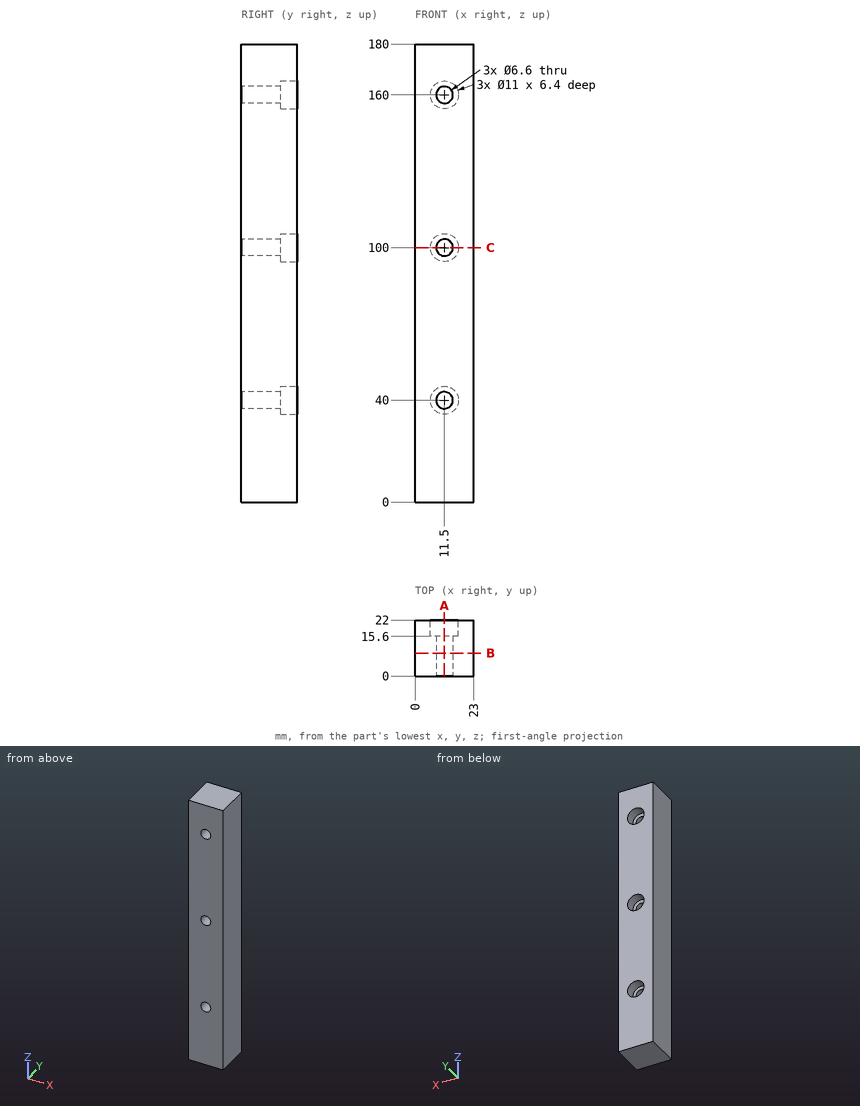
Design review of the part shown in the three views and the two pictorial views. Dimensions are in mm from the part's minimum x, y and z. Give positions to 0.01 mm unless a question says otherwise; leave off trailing zeros. Write each loop counter-clockwise with the first axis right and the second up, starting at its lowest first coordinate (ties: lowest second). Pieces come first, ordered by that corner, then holes. Notation, with made-up numbers: (70.5, 35.5) - (125.5, 35.5) arc R29 ccw to (125.5, 55.5) - close; hole circle Ø6 at (55.25, 61). An arc over 180 degrees is marked (long way). Return JSON: item names as keys, results as strings. Group by question number.
(1) We need section A-A, the plane x = 11.5. Give the boundary of the cut face in (y, z), then the cut area to 3 significant figures.
(2) Insertion check: pin 1 (10 mm diameter, centred on y = 14, z = 109, fed in from -X); pin 2 (5.5 mm diameter, centred on x = 11.5, z = 40, fed in from -Y); pin 3 (10.5 mm diameter, centred on x = 11.5, z = 160, fed in from +Y). Each pin has a flat end and moves straight along its axis. Give the tip position at first contact, or say it passes through.
(3) To check wall thickness, follow probe 1 along Z at (x, y) = (11.5, 12); probe 2 along Z at (x, y) = (11.5, 20); probe 3 along X at (y, z) = (19.75, 100). State the ranges of each line that lie inside material, in increasing order.
(4) We need section C-C, the plane z = 100. Give the boundary of the cut face in (x, y), then the cut area to 3 significant figures.
(5) We need section B-B, the plane y = 9. Give the boundary of the cut face in (x, z), then the cut area to 3 significant figures.
Reported:
{
 "1": {"outline": "(0, 0) - (22, 0) - (22, 34.5) - (15.6, 34.5) - (15.6, 36.7) - (0, 36.7) - close; (0, 43.3) - (15.6, 43.3) - (15.6, 45.5) - (22, 45.5) - (22, 94.5) - (15.6, 94.5) - (15.6, 96.7) - (0, 96.7) - close; (0, 103.3) - (15.6, 103.3) - (15.6, 105.5) - (22, 105.5) - (22, 154.5) - (15.6, 154.5) - (15.6, 156.7) - (0, 156.7) - close; (0, 163.3) - (15.6, 163.3) - (15.6, 165.5) - (22, 165.5) - (22, 180) - (0, 180) - close", "area": "3,440 mm2"},
 "2": {"pin 1": "stops at x = 0", "pin 2": "passes through", "pin 3": "stops at y = 15.6"},
 "3": {"probe 1": "z = 0 to 36.7, 43.3 to 96.7, 103.3 to 156.7, 163.3 to 180", "probe 2": "z = 0 to 34.5, 45.5 to 94.5, 105.5 to 154.5, 165.5 to 180", "probe 3": "x = 0 to 6, 17 to 23"},
 "4": {"outline": "(0, 0) - (8.2, 0) - (8.2, 15.6) - (6, 15.6) - (6, 22) - (0, 22) - close; (14.8, 0) - (23, 0) - (23, 22) - (17, 22) - (17, 15.6) - (14.8, 15.6) - close", "area": "333 mm2"},
 "5": {"outline": "(0, 0) - (23, 0) - (23, 180) - (0, 180) - close; hole circle Ø6.6 at (11.5, 40); hole circle Ø6.6 at (11.5, 100); hole circle Ø6.6 at (11.5, 160)", "area": "4,040 mm2"}
}
